The drawing under review shows one solid part. Ordinate dimensions are in mm from its lowest x, y, z. Coordinates: 2 decimals unless noted, no trailing zeros. Loops run counter-clockwise (first coordinate to the right, second up) from the corner with the lowest first, then second, coordinate; pieces in that order, holes last. Notation, with made-up numbers: M 28.25,-31.5 L 56.25,-31.5 A7 ccw 56.25,-23.5 Z; hole C 55.5,58 d6. An arc over 180 degrees is marked long. Use one line per item in the form item = value.
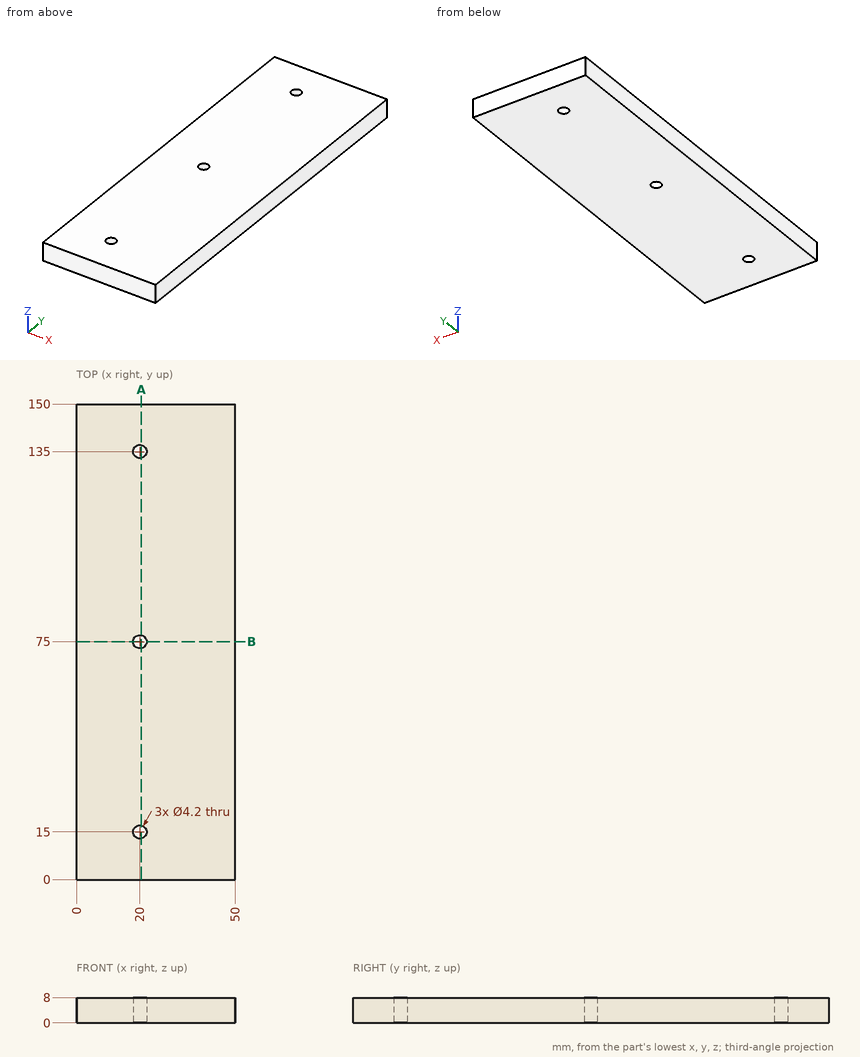
1. For pin 1 Ø4 at (y, z) = (77, 5.5) entering from -X; pin 2 Ø4 at (x, y) = (20, 75) entering from +Z, all flat-tipped, find the tip position at first contact; note any pin that passes through.
Computed values:
pin_1 = 0
pin_2 = through
2. Consider section B-B on y = 75. Write out the cut boundary in (x, z).
Computed values:
outline = M 0,0 L 17.9,0 L 17.9,8 L 0,8 Z; M 22.1,0 L 50,0 L 50,8 L 22.1,8 Z
3. Wall thickness on line 1 along Y through (x, z) = (20, 3.5); line 2 along X through (y, z) = (135, 4.75); line 3 along Y through (x, z) = (19, 5): over which ranges is each line inside the solid? List them lowest first. Write a range as from..to.
Computed values:
line_1 = 0..12.9, 17.1..72.9, 77.1..132.9, 137.1..150
line_2 = 0..17.9, 22.1..50
line_3 = 0..13.15, 16.85..73.15, 76.85..133.15, 136.85..150
4. Consider section A-A on x = 20.5. Write out the cut boundary in (y, z), plus the area to 3 significant figures.
Computed values:
outline = M 0,0 L 12.96,0 L 12.96,8 L 0,8 Z; M 17.04,0 L 72.96,0 L 72.96,8 L 17.04,8 Z; M 77.04,0 L 132.96,0 L 132.96,8 L 77.04,8 Z; M 137.04,0 L 150,0 L 150,8 L 137.04,8 Z
area = 1,100 mm2
